Work out the finished part from the listing and answer in its coordinate system (mm). A direction names the side the tool comes from. Round coordinates to 2 decimals unless told otherwise and drop trailing zeros. Write each loop counter-clockwise with the first axis right and the second up, starting at its lowest first coordinate (ties: lowest second). Pieces come first, ordered by that corner, then holes. Notation, with made-up numbers: (31.5, -9.5) - (84.5, -9.5) arc R6 cw to (84.5, -1.5) - close; hole circle Ø7 at (64.5, 43). An arc over 180 degrees is marked (long way). Answer as a JSON object with one key per item and string values.
```python
from build123d import *

# Parameters (mm, degrees)
SKETCH1_R           = 11
BOSS_EXTRUDE1_DEPTH = 8
SKETCH2_R           = 8
BOSS_EXTRUDE2_DEPTH = 10
BOSS_EXTRUDE3_START = 10
SKETCH3_R           = 8
BOSS_EXTRUDE3_DEPTH = 10
CHAMFER1_SIZE       = 1


with BuildPart() as part:
    # Sketch1 → Boss-Extrude1 (new body)
    with BuildSketch(Plane.XY):
        Circle(SKETCH1_R)
    extrude(amount=BOSS_EXTRUDE1_DEPTH)

    # Sketch2 → Boss-Extrude2 (add)
    with BuildSketch(Plane.XY.offset(8)):
        Circle(SKETCH2_R)
    extrude(amount=BOSS_EXTRUDE2_DEPTH)

    # Sketch3 → Boss-Extrude3 (add)
    with BuildSketch(Plane(origin=(0, 0, 0), x_dir=(-1, 0, 0), z_dir=(0, 0, -1)).offset(BOSS_EXTRUDE3_START)):
        with Locations(Location((0, 0, 0), (0, 0, 180))):
            Circle(SKETCH3_R)
    extrude(amount=-BOSS_EXTRUDE3_DEPTH)

    # Chamfer1
    chamfer1_edges = [part.edges().sort_by_distance(p)[0] for p in [
        (-8, 0, -10),
        (-8, 0, 18),
    ]]
    chamfer(chamfer1_edges, length=CHAMFER1_SIZE)


solid = part.part
```
Item 1: For faces 1 (the cylindrical face through (-2.38, -10.74, 3.94)), 2 (the cylindrical face through (-1.73, 7.81, -4.56)), 3 (the flat face through (-2, -8, 8)), determine the directions among +Z, -Z, +X, -X, +Y, -Y from which every point of the face is accessible in a straight line to the end or side of a thin tool.
Results found:
{"face 1": "+Z, -Z", "face 2": "-Z", "face 3": "+Z"}
Item 2: Consider line 1 along Z through (x, y) = (-8.75, -5.5); line 2 along Y through (x, z) = (0, 9.5); line 3 along Y through (x, z) = (-0.25, 5). Determine where each line is inside the solid, lowest interval first.
Results found:
{"line 1": "0 to 8", "line 2": "-8 to 8", "line 3": "-11 to 11"}
Item 3: A cutting plane is placed at D-D (y = 8.5). Write down the section's boundary in (x, z).
Results found:
{"outline": "(-6.98, 0) - (6.98, 0) - (6.98, 8) - (-6.98, 8) - close"}
Item 4: A cutting plane is placed at C-C (z = -0.5). Write down the section's boundary in (x, y).
Results found:
{"outline": "circle Ø16 at (0, 0)"}
Item 5: Each of these flat-tipped pins is pushed along its axis until it touches: P1, Ø3, axis at x = 4.5, z = 4.5, coming from the -Y side; P2, Ø8, axis at x = 7, z = 3.5, coming from the +Y side; P3, Ø10, axis at y = 3, z = 10.5, coming from the +X side; P4, Ø2, axis at x = -4.5, z = 14, coming from the +Y side. Where does it stop, or does it pass through?
Results found:
{"P1": "y = -10.58", "P2": "y = 10.58", "P3": "x = 11", "P4": "y = 7.19"}
Item 6: A cutting plane is placed at A-A (x = 0). Write down the section's boundary in (y, z), and give its area (3 significant figures).
Results found:
{"outline": "(-11, 0) - (-8, 0) - (-8, -9) - (-7, -10) - (7, -10) - (8, -9) - (8, 0) - (11, 0) - (11, 8) - (8, 8) - (8, 17) - (7, 18) - (-7, 18) - (-8, 17) - (-8, 8) - (-11, 8) - close", "area": "494 mm²"}
